Here's the drawing with two shaded views (mm, measured from the low corner). I have some questions. A direction names the side the tool comes from. Coordinates: 2 decimals unless noted, no trailing zeros. Write each loop counter-clockwise with the first axis right and the second up, starting at its lowest first coordinate (ties: lowest second). Pieces come first, ordered by that corner, then holes.
Item 1: If we section it at A-A (z = 30): Please give me the cut outline in (x, y), then the cut area to 3 significant figures.
Item 2: If we section it at B-B (x = 40): Please give me the cut outline in (y, z), then the cut area to 3 significant figures.
Item 3: If we section it at C-C (z = 44): Please give me the cut outline in (x, y), then the cut area to 3 significant figures.
Item 4: If we section it at D-D (y = 52.5): Please give me the cut outline in (x, z).
Item 5: If I drill on line 1 (Y direction, x = 10.5, z = 24.5); line 2 (Y direction, x = 59.5, z = 5.5); line 3 (Z direction, x = 9.5, y = 39.5), over which ranges is the centre line in solid material (lowest first)?
Item 6: I'm going to push flat-ended pins straight in: pin 1 Ø4 at (x, z) = (68, 41) entering from -Y; pin 2 Ø12 at (x, z) = (55.5, 12.5) entering from -Y; pin 3 Ø5 at (x, y) = (42.5, 9) entering from +Z. Where does each tip first touch, or does it pass through?
Item 7: For the marked faces 1, 2 and 3, which set-ups out of +Z, -Z, +X, -X, +Y, -Y let a thin tool reach every point of the face, with its end or its side?
Item 8: We'd pull the mould along Y, two halves only. Please class the marked faces 4, 5, 6 and 7: +Y half, -Y half, draft (parallel to the pull), parting line (faces both ways), or undercut.
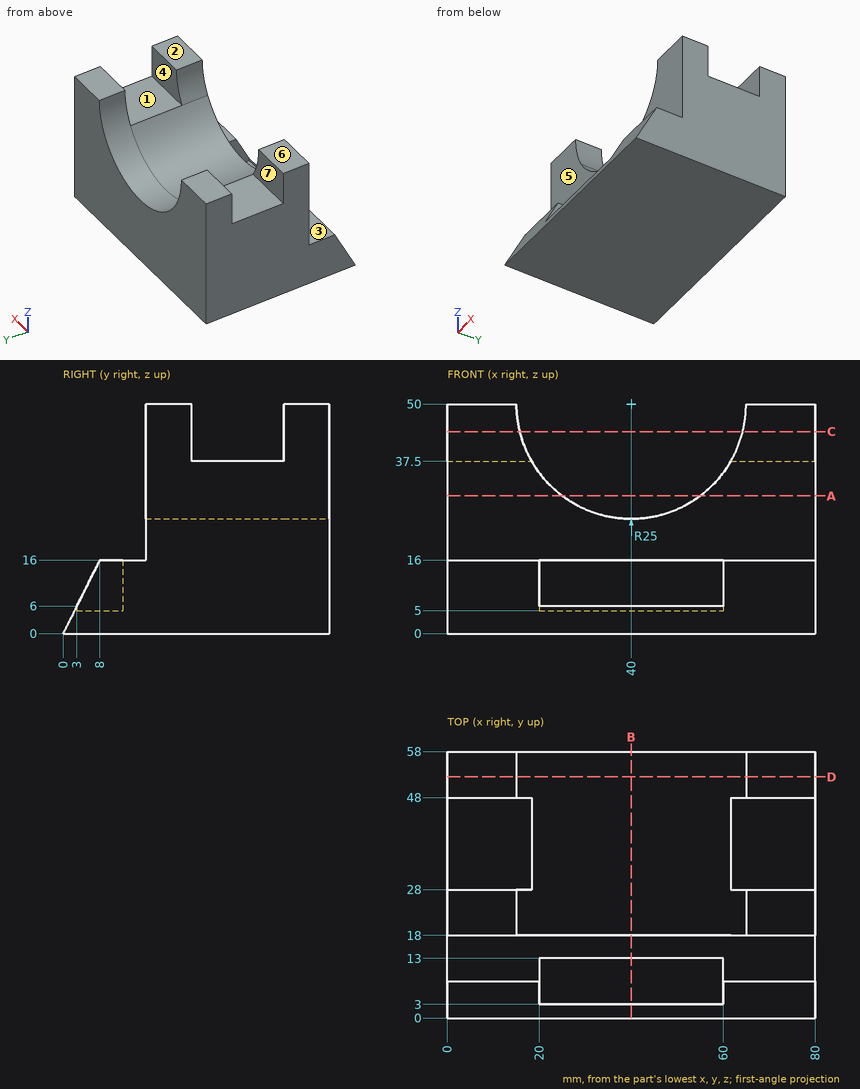
Answer list:
1. outline: (0, 18) - (25, 18) - (25, 58) - (0, 58) - close; (55, 18) - (80, 18) - (80, 58) - (55, 58) - close
1. area: 2,000 mm2
2. outline: (0, 0) - (58, 0) - (58, 25) - (18, 25) - (18, 16) - (13, 16) - (13, 5) - (3, 5) - (3, 6) - close
2. area: 1,140 mm2
3. outline: (0, 18) - (15.73, 18) - (15.73, 28) - (0, 28) - close; (0, 48) - (15.73, 48) - (15.73, 58) - (0, 58) - close; (64.27, 18) - (80, 18) - (80, 28) - (64.27, 28) - close; (64.27, 48) - (80, 48) - (80, 58) - (64.27, 58) - close
3. area: 629 mm2
4. outline: (0, 0) - (80, 0) - (80, 50) - (65, 50) arc R25 cw to (15, 50) - (0, 50) - close
5. line 1: y = 18 to 58
5. line 2: y = 2.75 to 3, 13 to 58
5. line 3: z = 0 to 37.5
6. pin 1: stops at y = 18
6. pin 2: stops at y = 4.27
6. pin 3: stops at z = 5
7. face 1: +Z, +X, -X
7. face 2: +Z, +X, -X, +Y, -Y
7. face 3: +Z, +X, -X, -Y
8. face 4: undercut
8. face 5: -Y half
8. face 6: draft
8. face 7: undercut
